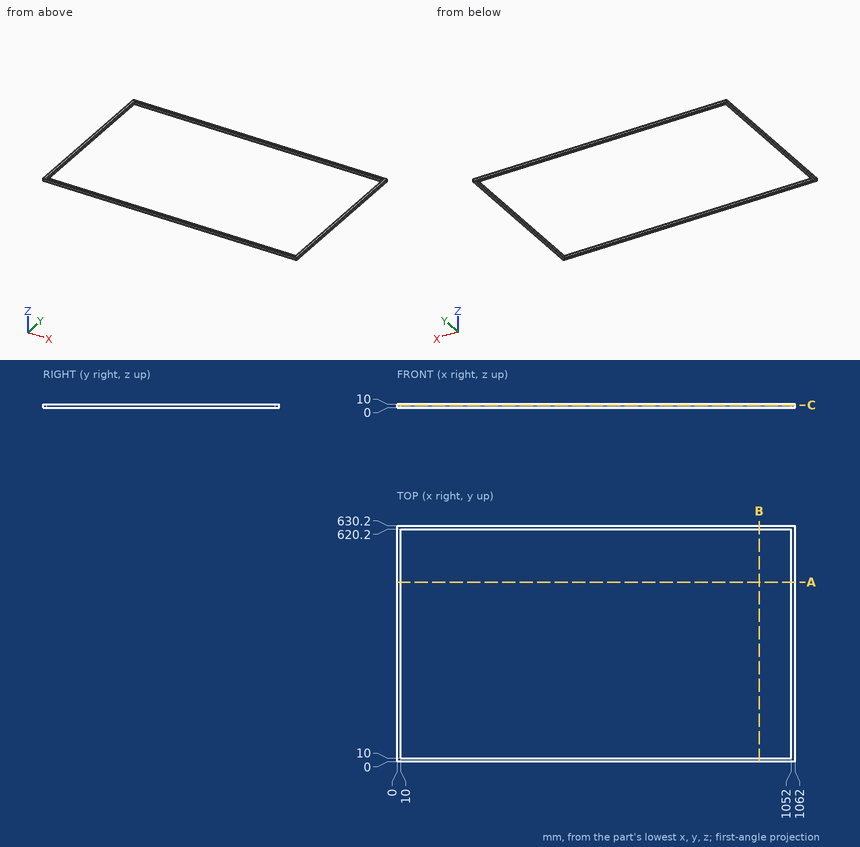
Geometry: see drawing. Coordinates: mm, zero at the bounding-box minimum. Coordinates: 2 decimals unless noted, no trailing zeros. Loops run counter-clockwise (first coordinate to the right, second up) from the corner with the lowest first, then second, coordinate; pieces in that order, holes last. Notation, with made-up numbers: M -22.75,4.5 L 33.25,4.5 A25 cw 33.25,27.5 Z; hole C 55,40 d9. An arc over 180 degrees is marked long. Put each result on its own line as item: value. Start each with the question number.
1) Cut plane A-A on y = 480. Return the cut outline in (x, z), then the cut area to 3 significant figures.
2) Cut plane C-C on z = 7. Return the cut outline in (x, y), then the cut area to 3 significant figures.
3) Cut plane B-B on x = 966.5. Return the cut outline in (y, z), then the cut area to 3 significant figures.
4) Ray query, L1, parallel to X at y = 475, z = 1.5; L2, parallel to Y at x = 386, z = 3.75. Return the intervals inside material, ascending. Write a range as from..to.
The answers:
1. outline: M 0,0 L 10,0 L 10,10 L 0,10 Z; M 1052,0 L 1062,0 L 1062,10 L 1052,10 Z
1. area: 200 mm²
2. outline: M 0,0 L 1062,0 L 1062,630.2 L 0,630.2 Z; hole M 10,10 L 1052,10 L 1052,620.2 L 10,620.2 Z
2. area: 33,400 mm²
3. outline: M 0,0 L 10,0 L 10,10 L 0,10 Z; M 620.2,0 L 630.2,0 L 630.2,10 L 620.2,10 Z
3. area: 200 mm²
4. L1: x = 0..10, 1052..1062
4. L2: y = 0..10, 620.2..630.2
